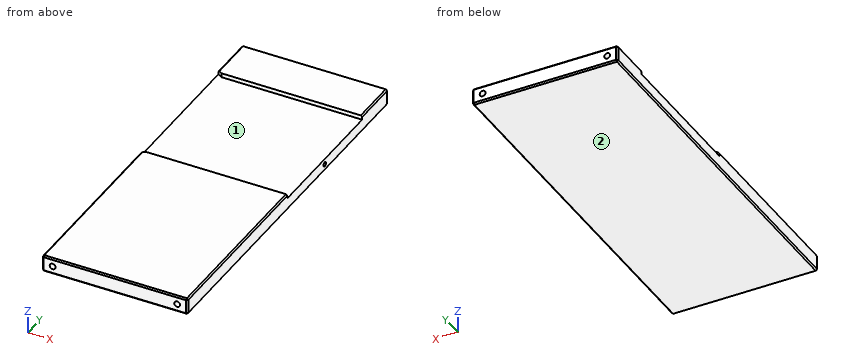
from build123d import *

# Parameters (mm, degrees)
SKETCH_1_W                  = 105
SKETCH_1_H                  = 270
EXTRUDE_1_DEPTH             = 12
SKETCH_2_W                  = 3
SKETCH_2_H                  = 101
CUT_EXTRUDE_1_DEPTH         = 172.446784747
HOLE_WIZARD_M5_1_AT_2_COUNT = 2
HOLE_WIZARD_M5_1_AT_2_PITCH = 90
CHAMFER_1_SIZE              = 1
CHAMFER_2_SIZE              = 2
CHAMFER_2_SIZE2             = 3.464101615
HOLE_WIZARD_M4_1_D          = 3.3
HOLE_WIZARD_M4_1_DEPTH      = 10.1
HOLE_WIZARD_M4_1_TIP        = 0.991420021


with BuildPart() as part:
    # 草图1 → 凸台-拉伸1 (new body)
    with BuildSketch(Plane.XY):
        Rectangle(SKETCH_1_W, SKETCH_1_H)
    extrude(amount=EXTRUDE_1_DEPTH)

    # 草图2 → 切除-拉伸1 (cut, through all)
    with BuildSketch(Plane(origin=(52.5, 0, 0), x_dir=(0, 0, -1), z_dir=(1, 0, 0))):
        with Locations((-10.5, 50)):
            Rectangle(SKETCH_2_W, SKETCH_2_H)
    extrude(amount=-CUT_EXTRUDE_1_DEPTH, mode=Mode.SUBTRACT)

    # 草图4 → M5 螺纹孔1 (revolve, cut)
    with BuildSketch(Plane(origin=(-45, -135, 6), x_dir=(0, 0, -1), z_dir=(1, 0, 0))):
        Polygon((0, 0), (0, 13.6618073), (2.1, 12.4), (2.1, 0), align=None)
    hole_wizard_m5_1 = revolve(axis=Axis((-45, -141.35, 6), (0, 1, 0)), mode=Mode.SUBTRACT)

    # M5 螺纹孔1 at 2: M5 螺纹孔1 ×2
    with Locations(*[(i * HOLE_WIZARD_M5_1_AT_2_PITCH, 0, 0) for i in range(1, HOLE_WIZARD_M5_1_AT_2_COUNT)]):
        add(hole_wizard_m5_1, mode=Mode.SUBTRACT)

    # 镜向1: M5 螺纹孔1 across plane
    add(hole_wizard_m5_1.mirror(Plane.ZX), mode=Mode.SUBTRACT)

    # 镜向1 copy 1 sketch → 镜向1 copy 1 (revolve, cut)
    with BuildSketch(Plane(origin=(45, 135, 6), x_dir=(0, 0, -1), z_dir=(1, 0, 0))):
        Polygon((0, 0), (0, -13.6618073), (2.1, -12.4), (2.1, 0), align=None)
    revolve(axis=Axis((45, 141.35, 6), (0, 1, 0)), mode=Mode.SUBTRACT)

    # 倒角1
    chamfer_1_edges = [part.edges().sort_by_distance(p)[0] for p in [
        (-52.5, 117.75, 12),
        (0, -135, 12),
        (52.5, 117.75, 12),
        (-52.5, -67.75, 12),
        (52.5, -67.75, 12),
        (0, -135, 0),
        (-52.5, 0, 0),
        (0, 135, 0),
        (52.5, 0, 0),
        (0, 135, 12),
        (52.5, -135, 6),
        (-52.5, -135, 6),
        (-52.5, 135, 6),
        (52.5, 135, 6),
    ]]
    chamfer(chamfer_1_edges, length=CHAMFER_1_SIZE)

    # 倒角2
    chamfer_2_edges = [part.edges().sort_by_distance(p)[0] for p in [
        (-52.5, -0.5, 10),
        (-52.5, 100.5, 10),
    ]]
    chamfer_2_side = [part.faces().sort_by_distance(p)[0] for p in [
        (-52.5, -4.075867635, 5.673930589),
    ]]
    chamfer(chamfer_2_edges, length=CHAMFER_2_SIZE, length2=CHAMFER_2_SIZE2, reference=chamfer_2_side[0])

    # M4 螺纹孔1
    with Locations(Plane(origin=(52.5, 0, 0), x_dir=(0, 0, -1), z_dir=(1, 0, 0))):
        with Locations((-5, 50)):
            Hole(HOLE_WIZARD_M4_1_D / 2, depth=HOLE_WIZARD_M4_1_DEPTH)
            with Locations((0, 0, -(HOLE_WIZARD_M4_1_DEPTH + HOLE_WIZARD_M4_1_TIP / 2))):  # 118° drill point
                Cone(0, HOLE_WIZARD_M4_1_D / 2, HOLE_WIZARD_M4_1_TIP, mode=Mode.SUBTRACT)


solid = part.part
Input: part model. Units: mm. Frame: model coordinates. Face numbers are marked on the shaded views. Coordinates: 2 decimals unless noted, no trailing zeros. Loops run counter-clockwise (first coordinate to the right, second up) from the corner with the lowest first, then second, coordinate; pieces in that order, holes last. Notation, with made-up numbers: (26, 48.5) -> (62, 48.5) arc R27 ccw to (62, 74.5) -> close; hole circle Ø8 at (85, 42). An arc over 180 degrees is marked (long way). Write each question's results on one line, items separated by ' | '. Start each with the question number.
Q1. Section B-B, the plane y = 3.5. Return the cut outline in (x, z), plus the area to 3 significant figures.
Q2. Section A-A, the plane x = 34. Return the cut outline in (y, z).
Q3. Ray query, line 1 (Z direction, x = -45, y = -130); line 2 (Z direction, x = 48, y = 50); line 3 (Y direction, x = -41, z = 10). Return the intervals inside material, ascending. Write a range as from..to.
Q4. Pull-direction query (Y, two-part tool) for the marked faces 1 and 2; classes: released by +Y, released by -Y, zero draft, split by the parting line, or undercut.
Q5. Pin query (flat end, axial travel): pin 1 (2.5 mm diameter, centred on y = 50, z = 5, fed in from +X); pin 2 (3.5 mm diameter, centred on x = 45, z = 6, fed in from +Y); pin 3 (6 mm diameter, centred on x = 9, y = 35, fed in from +Z). Return the tip coordinate at first contact, or that it passes through.
Found:
1) outline: (-52.5, 1) -> (-51.5, 0) -> (51.5, 0) -> (52.5, 1) -> (52.5, 9) -> (-52.5, 9) -> close | area: 944 mm2
2) outline: (-135, 1) -> (-134, 0) -> (134, 0) -> (135, 1) -> (135, 11) -> (134, 12) -> (100.5, 12) -> (100.5, 9) -> (-0.5, 9) -> (-0.5, 12) -> (-134, 12) -> (-135, 11) -> close
3) line 1: 0..3.9, 8.1..12 | line 2: 0..3.35, 6.65..9 | line 3: -135..-0.5, 100.5..135
4) face 1: undercut | face 2: zero draft
5) pin 1: x = 42.16 | pin 2: y = 122.39 | pin 3: z = 9
